Can you work these out from the model? Positions are in its coordinate system, mm. Face numbers are marked on the shaded views. A direction names the side the tool comes from. Give positions to 0.01 mm unless a question says otherwise; leave off trailing zeros. Loops run counter-clockwise (first coordinate to the right, second up) from the corner with the lowest first, then second, coordinate; pieces in that order, holes last.
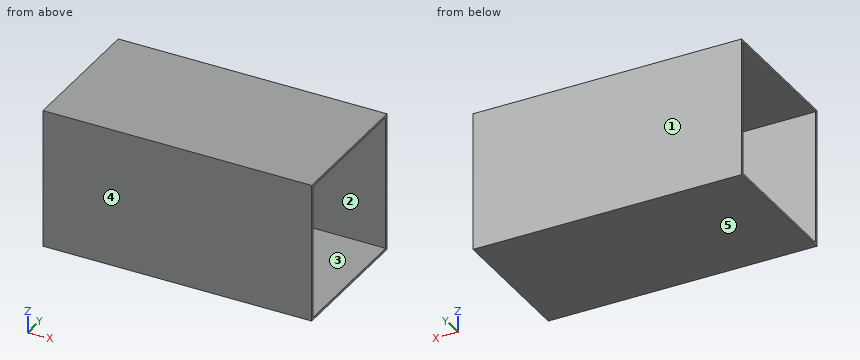
from build123d import *

# Parameters (mm, degrees)
SKETCH1_W           = 466
SKETCH1_H           = 466
SKETCH1_W_2         = 450
SKETCH1_H_2         = 450
BOSS_EXTRUDE1_DEPTH = 900


with BuildPart() as part:
    # Sketch1 → Boss-Extrude1 (new body)
    with BuildSketch(Plane(origin=(0, 0, 0), x_dir=(0, 0, -1), z_dir=(1, 0, 0))):
        Rectangle(SKETCH1_W, SKETCH1_H)
        Rectangle(SKETCH1_W_2, SKETCH1_H_2, mode=Mode.SUBTRACT)
    extrude(amount=BOSS_EXTRUDE1_DEPTH)


solid = part.part
(1) Thinking about a two-plate mould opening in Z: for the marked faces 3, 4 and 5, which applies, pulls with the +Z half, pulls with the -Z half, needs draft (parallel to the pull), parting line crosses it, or undercut?
Returned:
face 3: undercut
face 4: needs draft
face 5: pulls with the -Z half
(2) Suppose I cut it at A-A on x = 301. List the corners of the cut face in (y, z) for me, plus the area to 3 significant figures.
Returned:
outline: (-233, -233) - (233, -233) - (233, 233) - (-233, 233) - close; hole (-225, -225) - (225, -225) - (225, 225) - (-225, 225) - close
area: 14,700 mm2
(3) Suppose I cut it at B-B on y = 185.5. List the corners of the cut face in (x, z) for me.
Returned:
outline: (0, -233) - (900, -233) - (900, -225) - (0, -225) - close; (0, 225) - (900, 225) - (900, 233) - (0, 233) - close
(4) Which directions (+Z, -Z, +X, -X, +Y, -Y) give clear straight access to the entire face, cutting with the end or side of a thin tool? Please do the marked faces 1 and 2.
Returned:
face 1: +Z, -Z, +X, -X, +Y
face 2: +X, -X
(5) Please list where this line runs through material, in increasing order: probe 1 along Z at (x, y) = (393.5, 142).
Returned:
probe 1: z = -233 to -225, 225 to 233
